Check sheet for the drawn part. Datum: minimum x, y, z corner. Units: mm. Coordinates: 2 decimals unless noted, no trailing zeros. Order: outer loops, then holes, each group sorted by start corner. A loop starts at its lowest first (then second) coordinate and runs counter-clockwise, first axis right, second up. Notation, with made-up numbers: M 40.25,-15.5 L 66.25,-15.5 A16 cw 66.25,1.5 Z; hole C 62.25,-14 d4. An arc over 180 degrees is marked long. Answer in a Markdown table with one row per item. Add a question column.
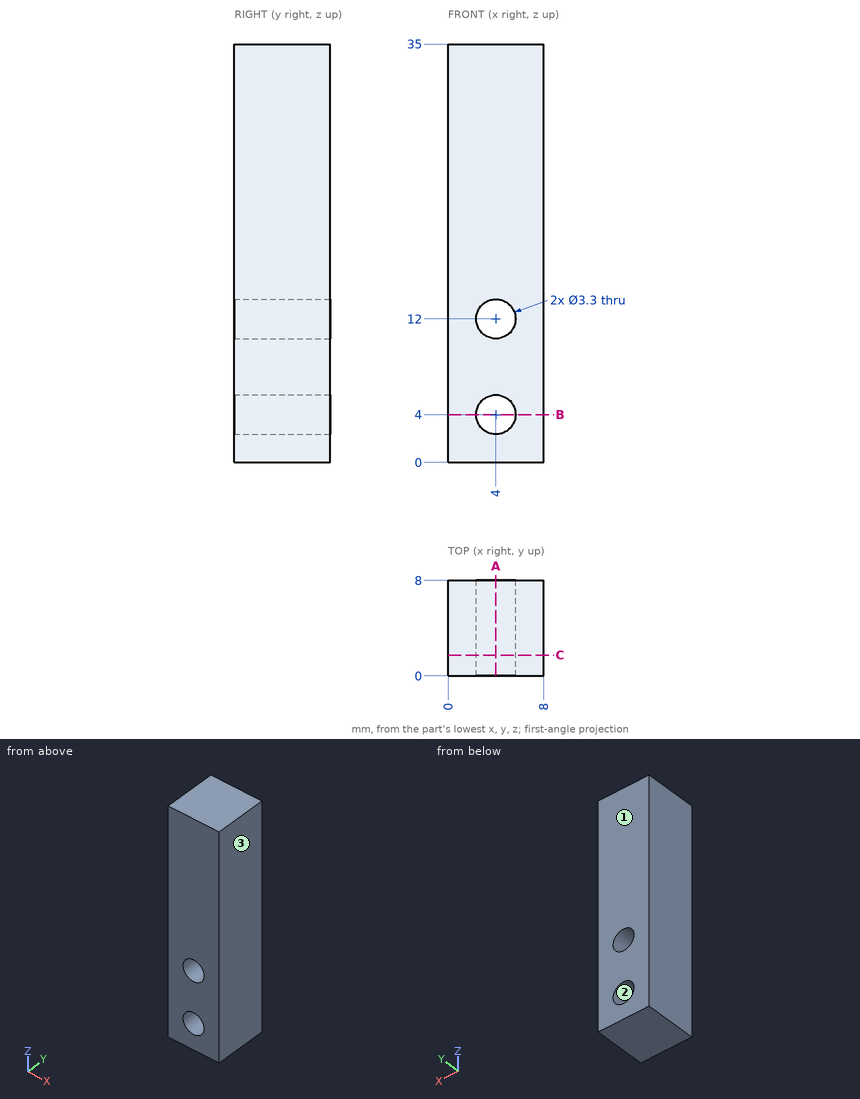
1. Section check C-C on y = 1.75. Enter the section's corners in (x, z).
2. Scan lines: line 1 (Z direction, x = 4, y = 6); line 2 (X direction, y = 5, z = 4); line 3 (Z direction, x = 2.5, y = 4.25). Record each from-to range of solid material in increasing order.
3. Section check B-B on z = 4. Enter the section's corners in (x, y), then the cut area to 3 significant figures.
4. Section check A-A on x = 4. Enter the section's corners in (y, z), then the cut area to 3 significant figures.
5. Release check for a two-part mould opening along X. For the marked faces 1, 2 and 3 record: released by +X, released by -X, zero draft, split by the parting line, or undercut.
Result sheet:
| question | item | result |
|---|---|---|
| 1 | outline | M 0,0 L 8,0 L 8,35 L 0,35 Z; hole C 4,4 d3.3; hole C 4,12 d3.3 |
| 2 | line 1 | 0 to 2.35, 5.65 to 10.35, 13.65 to 35 |
| 2 | line 2 | 0 to 2.35, 5.65 to 8 |
| 2 | line 3 | 0 to 3.31, 4.69 to 11.31, 12.69 to 35 |
| 3 | outline | M 0,0 L 2.35,0 L 2.35,8 L 0,8 Z; M 5.65,0 L 8,0 L 8,8 L 5.65,8 Z |
| 3 | area | 37.6 mm^2 |
| 4 | outline | M 0,0 L 8,0 L 8,2.35 L 0,2.35 Z; M 0,5.65 L 8,5.65 L 8,10.35 L 0,10.35 Z; M 0,13.65 L 8,13.65 L 8,35 L 0,35 Z |
| 4 | area | 227 mm^2 |
| 5 | face 1 | zero draft |
| 5 | face 2 | undercut |
| 5 | face 3 | released by +X |
